Source: CAD feature listing. Evaluate the final solid. Frame: model axes, mm. A direction names the side the tool comes from. Round coordinates to 2 decimals unless told otherwise and drop trailing zeros. Write each loop counter-clockwise with the first axis right and the second up, starting at its lowest first coordinate (ties: lowest second). Pieces come first, ordered by that corner, then holes. Notation, with made-up numbers: (-26, 16.25) - (9, 16.25) arc R10 ccw to (9, 23.25) - close; hole circle Ø6 at (54.25, 3). An arc over 180 degrees is marked (long way). Write item = value, one per line. Start each with the question number.
```python
from build123d import *

# Parameters (mm, degrees)
SKETCH1_W               = 20
SKETCH1_H               = 380
CUT_EXTRUDE1_DEPTH      = 344.613267812
CUT_EXTRUDE1_DEPTH_BACK = 344.613267812
SKETCH2_W               = 1
SKETCH2_H               = 30
CHAMFER1_SIZE           = 1.5
M12_TAPPED_HOLE1_D      = 10.2
M12_TAPPED_HOLE1_DEPTH  = 24
M12_TAPPED_HOLE1_TIP    = 3.064389157


with BuildPart() as part:
    # Sketch1 → Revolve1 (revolve)
    with BuildSketch(Plane.XY, mode=Mode.PRIVATE) as revolve1_sk:
        with Locations((-98.74611723, 135.337301587)):
            Rectangle(SKETCH1_W, SKETCH1_H)
    revolve(revolve1_sk.sketch.rotate(Axis((-88.74611723, 325.337301587, 0), (0, -1, 0)), 270), axis=Axis((-88.74611723, 325.337301587, 0), (0, -1, 0)))

    # Sketch2 → Cut-Extrude1 (cut, two sides: drawn at the far end of the back side and taken through both)
    with BuildSketch(Plane.XY.offset(-CUT_EXTRUDE1_DEPTH_BACK)):
        with Locations((-108.24611723, -29.662698413)):
            Rectangle(SKETCH2_W, SKETCH2_H)
        with Locations((-69.24611723, -29.662698413)):
            Rectangle(SKETCH2_W, SKETCH2_H)
    extrude(amount=CUT_EXTRUDE1_DEPTH + CUT_EXTRUDE1_DEPTH_BACK, mode=Mode.SUBTRACT)

    # Chamfer1
    chamfer1_edges = [part.edges().sort_by_distance(p)[0] for p in [
        (-88.74611723, -54.662698413, -20),
        (-88.74611723, 325.337301587, -20),
    ]]
    chamfer(chamfer1_edges, length=CHAMFER1_SIZE)

    # M12 Tapped Hole1
    with Locations(Plane(origin=(0, 325.337301587, 0), x_dir=(1, 0, 0), z_dir=(0, 1, 0))):
        with Locations((-88.74611723, 0)):
            Hole(M12_TAPPED_HOLE1_D / 2, depth=M12_TAPPED_HOLE1_DEPTH)
            with Locations((0, 0, -(M12_TAPPED_HOLE1_DEPTH + M12_TAPPED_HOLE1_TIP / 2))):  # 118° drill point
                Cone(0, M12_TAPPED_HOLE1_D / 2, M12_TAPPED_HOLE1_TIP, mode=Mode.SUBTRACT)


solid = part.part
```
(1) Section A-A (y = -19.5). Return the cut outline in (x, z) (3 decimals), plus the area to 3 significant figures.
(2) Contact query for flat-ended pins moving along their axis: P1, Ø1.1, axis at x = -69.5, z = 0.5, coming from the +Y side; P2, Ø6, axis at x = -76.5, y = 275, coming from the -Z side; P3, Ø8, axis at x = -82.5, y = 281, coming from the +Z side. Output: stop coordinate, or through.
(3) Pull-direction query (Y, two-part tool) for faces 1 (the cylindrical face through (-83.65, 313.17, -0.22)), 2 (the flat face through (-69.746, -30, 0)), 3 (the conical face through (-87.928, 298.805, 0.339)), 4 (the flat face through (-89, -54.663, 0)); classes: +Y half, -Y half, draft (parallel to the pull), parting line (faces both ways), or undercut.
(4) Section B-B (y = 199.5). Return the cut outline in (x, z), plus the area to 3 significant figures.
(5) Reachability of faces 5 (the flat face through (-107.746, -30, 0)), 6 (the flat face through (-85, 325.337, 4)) from +Z, -Z, +X, -X, +Y, -Y: full face, straight path, thin tool, end or side. Return the list, or none.
(6) Ray query, L1, parallel to X at y = 189, z = 0; L2, parallel to Z at x = -88.5, y = 169.5; L3, parallel to Z at x = -80.5, y = 289. Return the intervals inside material, ascending. Write a range as from..to.
Solution:
q1.outline = (-107.746, -6.245) arc R20 ccw to (-69.746, -6.245) - (-69.746, 6.245) arc R20 ccw to (-107.746, 6.245) - close
q1.area = 1,240 mm^2
q2.P1 = 325.13
q2.P2 = -17.73
q2.P3 = 19.87
q3.face_1 = draft
q3.face_2 = undercut
q3.face_3 = +Y half
q3.face_4 = -Y half
q4.outline = circle Ø40 at (-88.75, 0)
q4.area = 1,260 mm^2
q5.face_5 = +Z, -Z, -X
q5.face_6 = +Z, -Z, +X, -X, +Y
q6.L1 = -108.75..-68.75
q6.L2 = -20..20
q6.L3 = -18.22..18.22
